```python
from build123d import *

# Parameters (mm, degrees)
SKETCH_1_W                = 60
SKETCH_1_H                = 71
EXTRUDE_1_DEPTH           = 6
HOLE_WIZARD_M5_1_D        = 4.2
HOLE_WIZARD_6_0_6_1_D     = 6
SKETCH_7_W                = 6
SKETCH_7_H                = 71
EXTRUDE_2_DEPTH           = 40
HOLE_WIZARD_7_0_7_1_D     = 7
HOLE_WIZARD_7_0_7_1_DEPTH = 15
HOLE_WIZARD_7_0_7_1_TIP   = 2.103012167
CUT_EXTRUDE_1_DEPTH       = 81.375680401
CHAMFER_1_SIZE            = 10


with BuildPart() as part:
    # 草图1 → 凸台-拉伸1 (new body)
    with BuildSketch(Plane(origin=(0, 0, 0), x_dir=(0, 0, -1), z_dir=(1, 0, 0))):
        Rectangle(SKETCH_1_W, SKETCH_1_H)
    extrude(amount=EXTRUDE_1_DEPTH)

    # M5 螺纹孔1 (through all)
    with Locations(Plane(origin=(6, 0, 0), x_dir=(0, 0, -1), z_dir=(1, 0, 0))):
        with Locations((-15, 25.5), (-15, -6.5)):
            Hole(HOLE_WIZARD_M5_1_D / 2)

    # Ø6.0 (6) 直径孔1 (through all)
    with Locations(Plane.ZY):
        with Locations((-15, 10), (-15, -10)):
            Hole(HOLE_WIZARD_6_0_6_1_D / 2)

    # 草图7 → 凸台-拉伸2 (add)
    with BuildSketch(Plane.ZY):
        with Locations((-27, 0)):
            Rectangle(SKETCH_7_W, SKETCH_7_H)
    extrude(amount=EXTRUDE_2_DEPTH)

    # Ø7.0 (7) 直径孔1
    with Locations(Plane(origin=(0, 0, -30), x_dir=(-1, 0, 0), z_dir=(0, 0, -1))):
        with Locations((20, 10)):
            Hole(HOLE_WIZARD_7_0_7_1_D / 2, depth=HOLE_WIZARD_7_0_7_1_DEPTH)
            with Locations((0, 0, -(HOLE_WIZARD_7_0_7_1_DEPTH + HOLE_WIZARD_7_0_7_1_TIP / 2))):  # 118° drill point
                Cone(0, HOLE_WIZARD_7_0_7_1_D / 2, HOLE_WIZARD_7_0_7_1_TIP, mode=Mode.SUBTRACT)

    # 草图10 → 切除-拉伸1 (cut, through all)
    with BuildSketch(Plane(origin=(0, 0, -30), x_dir=(-1, 0, 0), z_dir=(0, 0, -1))):
        with BuildLine():
            ThreePointArc((1.997955587, -5.105508828), (20, -13.5), (38.002044413, -5.105508828))
            ThreePointArc((38.002044413, -5.105508828), (37.570645496, -0.174596643), (32.639733311, -0.60599556))
            ThreePointArc((32.639733311, -0.60599556), (20, -6.5), (7.360266689, -0.60599556))
            ThreePointArc((7.360266689, -0.60599556), (2.429354504, -0.174596643), (1.997955587, -5.105508828))
        make_face()
    extrude(amount=-CUT_EXTRUDE_1_DEPTH, mode=Mode.SUBTRACT)

    # 倒角1
    chamfer_1_edges = [part.edges().sort_by_distance(p)[0] for p in [
        (-40, -35.5, -27),
        (-40, 35.5, -27),
        (3, -35.5, 30),
        (3, 35.5, 30),
    ]]
    chamfer(chamfer_1_edges, length=CHAMFER_1_SIZE)


solid = part.part
```
Verification items for the finished model (mm, model axes). A direction names the side the tool comes from. Coordinates: 2 decimals unless noted, no trailing zeros. Order: outer loops, then holes, each group sorted by start corner. A loop starts at its lowest first (then second) coordinate and runs counter-clockwise, first axis right, second up. Notation, with made-up numbers: (-1.75, 53) -> (32.25, 53) arc R20 cw to (32.25, 87) -> close; hole circle Ø9 at (9, 23). An arc over 180 degrees is marked (long way). Put each result on its own line as item: value. Start each with the question number.
1) Cross-section at C-C (y = -10). Enter the section's corners in (x, z).
2) Material ranges on L1, parallel to Y at x = -20, z = -25.55; L2, parallel to Y at x = 4.25, z = 15; L3, parallel to Z at x = -9.5, y = -24.5, recorded low to high.
3) Go/stop test with flat-tipped pins: pin 1 (8 mm diameter, centred on x = -20, y = 10, fed in from +Z); pin 2 (4 mm diameter, centred on y = 25.5, z = 15, fed in from +X); pin 3 (2 mm diameter, centred on y = -19.5, z = 8.5, fed in from -X). Record where each tip stops, or that it passes through.
4) Tool access check on faces 5 (the cylindrical face through (-19.7, -13.5, -27)), 6 (the flat face through (-20, 0, -24)), 7 (the flat face through (3, 0, 30)). Record the directions out of +Z, -Z, +X, -X, +Y, -Y that give a thin tool (end or side, any length) a straight path to the whole face; none if there is none.
5) Cross-section at A-A (z = -15). Enter the section's corners in (x, y).
6) Release check for a two-part mould opening along X. For faces 1 (the cylindrical face through (-2.489, -0.126, -27.042)), 2 (the flat face through (6, 0, 0)), 3 (the flat face through (1, -35.5, -13)), 4 (the flat face through (-34.9, -30.6, -27)) record: pulls with the +X half, pulls with the -X half, needs draft (parallel to the pull), parting line crosses it, or undercut.
7) Cross-section at D-D (x = -12.5). Enter the section's corners in (y, z).
8) Cross-section at B-B (x = -20). Enter the section's corners in (y, z), plus the area to 3 significant figures.
Geometry check:
1. outline: (-40, -30) -> (-32.34, -30) -> (-32.34, -24) -> (-40, -24) -> close; (-7.66, -30) -> (6, -30) -> (6, -18) -> (0, -18) -> (0, -24) -> (-7.66, -24) -> close; (0, -12) -> (6, -12) -> (6, 30) -> (0, 30) -> close
2. L1: y = -35.5 to -13.5, -6.5 to 6.5, 13.5 to 35.5
2. L2: y = -35.5 to -8.6, -4.4 to 23.4, 27.6 to 35.5
2. L3: z = -30 to -24
3. pin 1: stops at z = -24
3. pin 2: passes through
3. pin 3: stops at x = 0
4. face 5: +Z, -Z
4. face 6: +Z, -X, +Y, -Y
4. face 7: +Z, +X, -X, +Y, -Y
5. outline: (0, -35.5) -> (6, -35.5) -> (6, -13) -> (0, -13) -> close; (0, -7) -> (6, -7) -> (6, 7) -> (0, 7) -> close; (0, 13) -> (6, 13) -> (6, 35.5) -> (0, 35.5) -> close
6. face 1: undercut
6. face 2: pulls with the +X half
6. face 3: needs draft
6. face 4: pulls with the -X half
7. outline: (-35.5, -30) -> (-12.27, -30) -> (-12.27, -24) -> (-35.5, -24) -> close; (-4.7, -30) -> (35.5, -30) -> (35.5, -24) -> (-4.7, -24) -> close
8. outline: (-35.5, -30) -> (-13.5, -30) -> (-13.5, -24) -> (-35.5, -24) -> close; (-6.5, -30) -> (6.5, -30) -> (6.5, -24) -> (-6.5, -24) -> close; (13.5, -30) -> (35.5, -30) -> (35.5, -24) -> (13.5, -24) -> close
8. area: 342 mm^2
